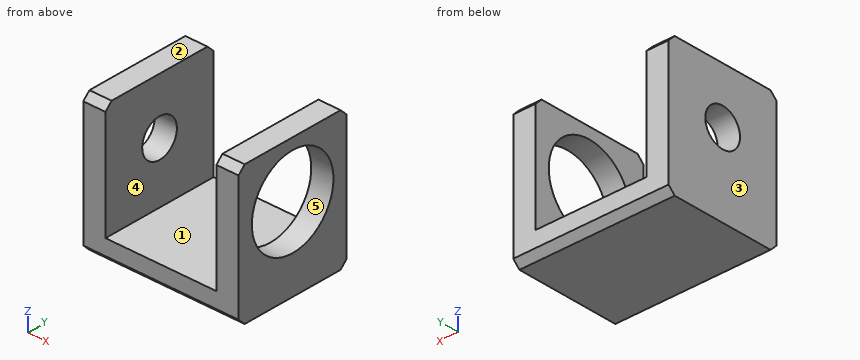
from build123d import *

# Parameters (mm, degrees)
EXTRUDE_1_DEPTH     = 26.5
CUT_EXTRUDE_2_REACH = 99.192
SKETCH_7_R          = 8.5
CUT_EXTRUDE_3_REACH = 92.257
SKETCH_8_R          = 20
CHAMFER_2_SIZE      = 3
CHAMFER_3_SIZE      = 3


with BuildPart() as part:
    # 草图1 → 凸台-拉伸1 (new, symmetric)
    with BuildSketch(Plane(origin=(0, 0, 0), x_dir=(1, 0, 0), z_dir=(0, 1, 0))):
        Polygon((0, 0), (0, 52), (50, 52), (50, 0), (60, 0), (60, 62), (-10, 62), (-10, 0), align=None)
    extrude(amount=EXTRUDE_1_DEPTH, both=True)

    # 草图7 → 切除-拉伸2 (cut, up to next)
    with BuildSketch(Plane.ZY.offset(10), mode=Mode.PRIVATE) as cut_extrude_2_sk1:
        with Locations((-25, 0)):
            Circle(SKETCH_7_R)
    cut_extrude_2_tool1 = extrude(cut_extrude_2_sk1.sketch, amount=-CUT_EXTRUDE_2_REACH, mode=Mode.PRIVATE) & part.part
    add(cut_extrude_2_tool1.solids().sort_by_distance((-10, 0, -25))[0], mode=Mode.SUBTRACT)

    # 草图8 → 切除-拉伸3 (cut, up to next)
    with BuildSketch(Plane.ZY.offset(-50), mode=Mode.PRIVATE) as cut_extrude_3_sk1:
        with Locations((-25, 0)):
            Circle(SKETCH_8_R)
    cut_extrude_3_tool1 = extrude(cut_extrude_3_sk1.sketch, amount=-CUT_EXTRUDE_3_REACH, mode=Mode.PRIVATE) & part.part
    add(cut_extrude_3_tool1.solids().sort_by_distance((50, 0, -25))[0], mode=Mode.SUBTRACT)

    # 倒角2
    chamfer_2_edges = [part.edges().sort_by_distance(p)[0] for p in [
        (25, 26.5, -62),
        (25, -26.5, -62),
    ]]
    chamfer(chamfer_2_edges, length=CHAMFER_2_SIZE)

    # 倒角3
    chamfer_3_edges = [part.edges().sort_by_distance(p)[0] for p in [
        (-5, -26.5, 0),
        (55, 26.5, 0),
        (-5, 26.5, 0),
        (55, -26.5, 0),
    ]]
    chamfer(chamfer_3_edges, length=CHAMFER_3_SIZE)


solid = part.part
Design review of the part built by this model. Coordinates are the model's own, in mm. Face numbers are marked on the shaded views. A direction names the side the tool comes from. Round coordinates to 2 decimals unless told otherwise and drop trailing zeros. Loops run counter-clockwise (first coordinate to the right, second up) from the corner with the lowest first, then second, coordinate; pieces in that order, holes last. Notation, with made-up numbers: M -15,1 L -2,1 A16 ccw -2,28 Z; hole C 88,35 d4. An arc over 180 degrees is marked long. Answer as a JSON object with one key per item and string values.
Item 1: We need section B-B on z = -25. Give the boundary of the cut face in (x, y), and give its area (3 significant figures).
Answer sheet:
{"outline": "M -10,-26.5 L 0,-26.5 L 0,-8.5 L -10,-8.5 Z; M -10,8.5 L 0,8.5 L 0,26.5 L -10,26.5 Z; M 50,-26.5 L 60,-26.5 L 60,-20 L 50,-20 Z; M 50,20 L 60,20 L 60,26.5 L 50,26.5 Z", "area": "490 mm^2"}
Item 2: We need section D-D on z = -7. Give the boundary of the cut face in (x, y).
Answer sheet:
{"outline": "M -10,-26.5 L 0,-26.5 L 0,26.5 L -10,26.5 Z; M 50,-26.5 L 60,-26.5 L 60,-8.72 L 50,-8.72 Z; M 50,8.72 L 60,8.72 L 60,26.5 L 50,26.5 Z"}
Item 3: We need section A-A on y = 0. Give the boundary of the cut face in (x, z), and give its area (3 significant figures).
Answer sheet:
{"outline": "M -10,-62 L 60,-62 L 60,-45 L 50,-45 L 50,-52 L 0,-52 L 0,-33.5 L -10,-33.5 Z; M -10,-16.5 L 0,-16.5 L 0,0 L -10,0 Z; M 50,-5 L 60,-5 L 60,0 L 50,0 Z", "area": "1,170 mm^2"}
Item 4: Wall thickness on L1, parallel to Y at x = 54.25, z = -25; L2, parallel to X at y = 7, z = -5; L3, parallel to Y at x = -7.5, z = -25: over which ranges is each line inside the solid? List them lowest first. Write a range as from..to.
Answer sheet:
{"L1": "y = -26.5..-20, 20..26.5", "L2": "x = -10..0, 50..60", "L3": "y = -26.5..-8.5, 8.5..26.5"}
Item 5: The part is to be moulded in two halves that separate along X. For the marked faces 3, 4 and 5, say which applies: pulls with the +X half, pulls with the -X half, needs draft (parallel to the pull), parting line crosses it, or undercut.
Answer sheet:
{"face 3": "pulls with the -X half", "face 4": "undercut", "face 5": "needs draft"}
Item 6: Clearance check with flat-ended pins moving along their axes: P1, Ø15.5, axis at y = -3, z = -25, coming from the +X side; P2, Ø6, axis at x = 36.5, y = 11, coming from the +Z side. State where each tip first meets the part, or that it passes through.
Answer sheet:
{"P1": "stops at x = 0", "P2": "stops at z = -52"}
Item 7: We need section C-C on y = 11. Give the boundary of the cut face in (x, z), and give its area (3 significant figures).
Answer sheet:
{"outline": "M -10,-62 L 60,-62 L 60,-41.7 L 50,-41.7 L 50,-52 L 0,-52 L 0,0 L -10,0 Z; M 50,-8.3 L 60,-8.3 L 60,0 L 50,0 Z", "area": "1,410 mm^2"}
Item 8: Machinability: for the marked faces 1 and 2, which of the approach directions +Z, -Z, +X, -X, +Y, -Y give a long, thin tool a straight path to every point of the face, cutting with its end or side? Answer none if there is none.
Answer sheet:
{"face 1": "+Z, +Y, -Y", "face 2": "+Z, +X, -X, +Y, -Y"}
